from build123d import *

# Parameters (mm, degrees)
SKETCH1_R           = 15
BOSS_EXTRUDE1_DEPTH = 15
CUT_EXTRUDE1_REACH  = 200.557
SKETCH6_W           = 73.144376366
SKETCH6_H           = 72.943161699
SKETCH6_W_2         = 11.5
SKETCH6_H_2         = 61
SKETCH6_W_3         = 13.06
SKETCH6_H_3         = 60.56
SKETCH6_W_4         = 7
SKETCH6_H_4         = 9
SKETCH7_W           = 22
SKETCH7_H           = 52
CUT_EXTRUDE2_DEPTH  = 10
FILLET1_R           = 1


with BuildPart() as part:
    # Sketch1 → Boss-Extrude1 (new body)
    with BuildSketch(Plane(origin=(0, 0, 0), x_dir=(1, 0, 0), z_dir=(0, 1, 0))):
        with BuildLine():
            Line((-110, -140), (80, -140))
            Line((80, -140), (80, 140))
            Line((80, 140), (-110, 140))
            ThreePointArc((-110, 140), (-140, 110), (-110, 80))
            Line((-110, 80), (-110, -80))
            ThreePointArc((-110, -80), (-140, -110), (-110, -140))
        make_face()
        with Locations(Location((-110, 110, 0), (0, 0, 270))):
            Circle(SKETCH1_R, mode=Mode.SUBTRACT)
        with Locations(Location((-110, -110, 0), (0, 0, 270))):
            Circle(SKETCH1_R, mode=Mode.SUBTRACT)
    boss_extrude1 = extrude(amount=BOSS_EXTRUDE1_DEPTH)

    # Mirror1: Boss-Extrude1 across plane
    add(boss_extrude1.mirror(Plane(origin=(0, 0, 0), x_dir=(0, 0, 1), z_dir=(1, 0, 0))))

    # Sketch6 → Cut-Extrude1 (cut, up to next)
    with BuildSketch(Plane(origin=(0, 15, 0), x_dir=(1, 0, 0), z_dir=(0, 1, 0)), mode=Mode.PRIVATE) as cut_extrude1_sk1:
        with Locations((0, -61.02841915)):
            Rectangle(SKETCH6_W, SKETCH6_H)
    cut_extrude1_tool1 = extrude(cut_extrude1_sk1.sketch, amount=-CUT_EXTRUDE1_REACH, mode=Mode.PRIVATE) & part.part
    # Sketch6 → Cut-Extrude1 (cut, up to next)
    with BuildSketch(Plane(origin=(0, 15, 0), x_dir=(1, 0, 0), z_dir=(0, 1, 0)), mode=Mode.PRIVATE) as cut_extrude1_sk2:
        with Locations((-15, 7)):
            Rectangle(SKETCH6_W_2, SKETCH6_H_2)
    cut_extrude1_tool2 = extrude(cut_extrude1_sk2.sketch, amount=-CUT_EXTRUDE1_REACH, mode=Mode.PRIVATE) & part.part
    # Sketch6 → Cut-Extrude1 (cut, up to next)
    with BuildSketch(Plane(origin=(0, 15, 0), x_dir=(1, 0, 0), z_dir=(0, 1, 0)), mode=Mode.PRIVATE) as cut_extrude1_sk3:
        Polygon((-0.14, 38), (-0.14, 44.06), (-29.63, 44.06), (-29.63, 46.06), (-48.5, 46.06), (-48.5, 36), (-29.63, 36), (-29.63, 38), align=None)
    cut_extrude1_tool3 = extrude(cut_extrude1_sk3.sketch, amount=-CUT_EXTRUDE1_REACH, mode=Mode.PRIVATE) & part.part
    # Sketch6 → Cut-Extrude1 (cut, up to next)
    with BuildSketch(Plane(origin=(0, 15, 0), x_dir=(1, 0, 0), z_dir=(0, 1, 0)), mode=Mode.PRIVATE) as cut_extrude1_sk4:
        Polygon((29.63, 36), (48.5, 36), (48.5, 46.06), (29.63, 46.06), (29.63, 44.06), (0.14, 44.06), (0.14, 38), (29.63, 38), align=None)
    cut_extrude1_tool4 = extrude(cut_extrude1_sk4.sketch, amount=-CUT_EXTRUDE1_REACH, mode=Mode.PRIVATE) & part.part
    # Sketch6 → Cut-Extrude1 (cut, up to next)
    with BuildSketch(Plane(origin=(0, 15, 0), x_dir=(1, 0, 0), z_dir=(0, 1, 0)), mode=Mode.PRIVATE) as cut_extrude1_sk5:
        with Locations((0.22, 7.22)):
            Rectangle(SKETCH6_W_3, SKETCH6_H_3)
    cut_extrude1_tool5 = extrude(cut_extrude1_sk5.sketch, amount=-CUT_EXTRUDE1_REACH, mode=Mode.PRIVATE) & part.part
    # Sketch6 → Cut-Extrude1 (cut, up to next)
    with BuildSketch(Plane(origin=(0, 15, 0), x_dir=(1, 0, 0), z_dir=(0, 1, 0)), mode=Mode.PRIVATE) as cut_extrude1_sk6:
        with Locations((15, 7)):
            Rectangle(SKETCH6_W_2, SKETCH6_H_2)
    cut_extrude1_tool6 = extrude(cut_extrude1_sk6.sketch, amount=-CUT_EXTRUDE1_REACH, mode=Mode.PRIVATE) & part.part
    # Sketch6 → Cut-Extrude1 (cut, up to next)
    with BuildSketch(Plane(origin=(0, 15, 0), x_dir=(1, 0, 0), z_dir=(0, 1, 0)), mode=Mode.PRIVATE) as cut_extrude1_sk7:
        with Locations((-36.69, 10.5)):
            Rectangle(SKETCH6_W_4, SKETCH6_H_4)
    cut_extrude1_tool7 = extrude(cut_extrude1_sk7.sketch, amount=-CUT_EXTRUDE1_REACH, mode=Mode.PRIVATE) & part.part
    # Sketch6 → Cut-Extrude1 (cut, up to next)
    with BuildSketch(Plane(origin=(0, 15, 0), x_dir=(1, 0, 0), z_dir=(0, 1, 0)), mode=Mode.PRIVATE) as cut_extrude1_sk8:
        with Locations((36.69, 10.5)):
            Rectangle(SKETCH6_W_4, SKETCH6_H_4)
    cut_extrude1_tool8 = extrude(cut_extrude1_sk8.sketch, amount=-CUT_EXTRUDE1_REACH, mode=Mode.PRIVATE) & part.part
    add(cut_extrude1_tool1.solids().sort_by_distance((0, 15, 61.028419))[0], mode=Mode.SUBTRACT)
    add(cut_extrude1_tool2.solids().sort_by_distance((-15, 15, -7))[0], mode=Mode.SUBTRACT)
    add(cut_extrude1_tool3.solids().sort_by_distance((-27.339883, 15, -41.03))[0], mode=Mode.SUBTRACT)
    add(cut_extrude1_tool4.solids().sort_by_distance((27.339883, 15, -41.03))[0], mode=Mode.SUBTRACT)
    add(cut_extrude1_tool5.solids().sort_by_distance((0.22, 15, -7.22))[0], mode=Mode.SUBTRACT)
    add(cut_extrude1_tool6.solids().sort_by_distance((15, 15, -7))[0], mode=Mode.SUBTRACT)
    add(cut_extrude1_tool7.solids().sort_by_distance((-36.69, 15, -10.5))[0], mode=Mode.SUBTRACT)
    add(cut_extrude1_tool8.solids().sort_by_distance((36.69, 15, -10.5))[0], mode=Mode.SUBTRACT)

    # Sketch7 → Cut-Extrude2 (cut)
    with BuildSketch(Plane.XZ):
        with Locations((49, -88.06497659)):
            Rectangle(SKETCH7_W, SKETCH7_H)
        with Locations((-49, -88.06497659)):
            Rectangle(SKETCH7_W, SKETCH7_H)
    extrude(amount=-CUT_EXTRUDE2_DEPTH, mode=Mode.SUBTRACT)

    # Fillet1
    fillet1_edges = [part.edges().sort_by_distance(p)[0] for p in [
        (60, 10, -88.06497659),
        (49, 10, -114.06497659),
        (38, 10, -88.06497659),
        (49, 10, -62.06497659),
        (60, 0, -88.06497659),
        (49, 0, -62.06497659),
        (38, 0, -88.06497659),
        (49, 0, -114.06497659),
        (-60, 10, -88.06497659),
        (-49, 10, -62.06497659),
        (-38, 10, -88.06497659),
        (-49, 10, -114.06497659),
        (-60, 0, -88.06497659),
        (-49, 0, -114.06497659),
        (-38, 0, -88.06497659),
        (-49, 0, -62.06497659),
    ]]
    fillet(fillet1_edges, radius=FILLET1_R)


solid = part.part
Input: part model. Units: mm. Frame: model coordinates. A direction names the side the tool comes from. Coordinates: 2 decimals unless noted, no trailing zeros. Order: outer loops, then holes, each group sorted by start corner. A loop starts at its lowest first (then second) coordinate and runs counter-clockwise, first axis right, second up. Notation, with made-up numbers: M -3.75,25 L 46.25,25 A33 cw 46.25,56 Z; hole C 61,73 d8. An arc over 180 degrees is marked long. Write item = value, one per line. Start each with the question number.
(1) Section B-B on z = 110. Output: boundary loops of the cut face in (x, y).
(2) Reachability of faces 4 (the flat face through (33, 0, -2)), 5 (the flat face through (-15, 8, -37.5)), 6 (the flat face through (49, 5, -114.065)) from +Z, -Z, +X, -X, +Y, -Y: full face, straight path, thin tool, end or side. Return the list, or none.
(3) First-contact query: P1, Ø2.5, axis at y = 6, z = -100.5, coming from the -X side; P2, Ø1, axis at y = 3, z = 30, coming from the -X side; P3, Ø1, axis at y = 8.5, z = 91.5, coming from the -X side. Flat tips, straight axial feed; report the tip coordinate or a pass-through.
(4) Section A-A on x = 14.5. Output: boundary loops of the cut face in (y, z), and give its area (3 significant figures).
(5) Pull-direction query (X, two-part tool) for faces 1 (the flat face through (33, 15, -2)), 2 (the cylindrical face through (124.643, 7.395, -113.252)), 3 (the cylindrical face through (-139.993, 7.395, 109.34)); classes: released by +X, released by -X, zero draft, split by the parting line, or undercut.
(6) Section D-D on z = -100.5. Output: boundary loops of the cut face in (x, y), and give its area (3 significant figures).
(7) Section C-C on y = 4.25. Give the number of separate pieces and of enclosed holes in the cut face, and give its area (3 significant figures).
(8) Line query: line 1 along X through (y, z) = (11.25, 110); line 2 along Z through (x, y) = (-1, 13.25); line 3 along X through (y, z) = (9, -110). Output: solid intervals per line, ascending. Write a range as [from, to].
Result set:
q1.outline = M -140,0 L -125,0 L -125,15 L -140,15 Z; M -95,0 L 95,0 L 95,15 L -95,15 Z; M 125,0 L 140,0 L 140,15 L 125,15 Z
q2.face_4 = +Z, -Z, +X, -X, -Y
q2.face_5 = +Y, -Y
q2.face_6 = -Y
q3.P1 = -138.84
q3.P2 = -110
q3.P3 = -134
q4.outline = M 0,-140 L 15,-140 L 15,-44.06 L 0,-44.06 Z; M 0,-38 L 15,-38 L 15,-37.5 L 0,-37.5 Z; M 0,23.5 L 15,23.5 L 15,24.56 L 0,24.56 Z; M 0,97.5 L 15,97.5 L 15,140 L 0,140 Z
q4.area = 2,100 mm²
q5.face_1 = zero draft
q5.face_2 = undercut
q5.face_3 = released by -X
q6.outline = M -138.46,0 L -121.61,0 L -121.61,15 L -138.46,15 Z; M -98.39,0 L -61,0 A1 ccw -60,1 L -60,9 A1 cw -59,10 L -39,10 A1 cw -38,9 L -38,1 A1 ccw -37,0 L 37,0 A1 ccw 38,1 L 38,9 A1 cw 39,10 L 59,10 A1 cw 60,9 L 60,1 A1 ccw 61,0 L 98.39,0 L 98.39,15 L -98.39,15 Z; M 121.61,0 L 138.46,0 L 138.46,15 L 121.61,15 Z
q6.area = 3,020 mm²
q7.separate_pieces = 1
q7.enclosed_holes = 14
q7.area = 53,700 mm²
q8.line_1 = [-140, -125], [-95, 95], [125, 140]
q8.line_2 = [-140, -44.06], [-38, -37.5], [23.06, 24.56], [97.5, 140]
q8.line_3 = [-140, -125], [-95, -60], [-38, 38], [60, 95], [125, 140]
